```python
from build123d import *

# Parameters (mm, degrees)
SHAFT_PROFILE_6_R        = 3
SHAFT_6X95_DEPTH         = 47.5
HEAD_PROFILE_10_R        = 5
HEAD_10X5_DEPTH          = 5
HEAD_EDGE_FILLETS_R0_5_R = 0.5


with BuildPart() as part:
    # Shaft Profile Ø6 → Shaft Ø6x95 (new, symmetric)
    with BuildSketch(Plane.XY):
        Circle(SHAFT_PROFILE_6_R)
    extrude(amount=SHAFT_6X95_DEPTH, both=True)

    # Head Profile Ø10 → Head Ø10x5 (add)
    with BuildSketch(Plane.XY.offset(47.5)):
        Circle(HEAD_PROFILE_10_R)
    head_10x5 = extrude(amount=-HEAD_10X5_DEPTH)

    # Head Mirror: Head Ø10x5 across plane
    add(head_10x5.mirror(Plane.XY))

    # Head Edge Fillets R0.5
    head_edge_fillets_r0_5_edges = [part.edges().sort_by_distance(p)[0] for p in [
        (-3, 0, -42.5),
        (-5, 0, -47.5),
        (-3, 0, 42.5),
        (-5, 0, 47.5),
    ]]
    fillet(head_edge_fillets_r0_5_edges, radius=HEAD_EDGE_FILLETS_R0_5_R)


solid = part.part
```
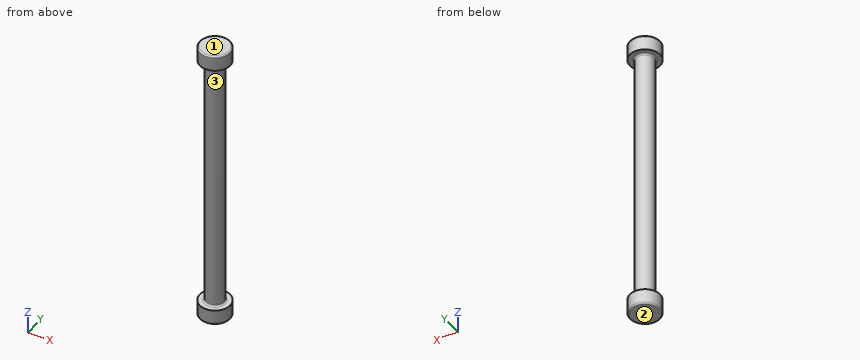
Here's how the part is built. I have some questions about the finished solid (model axes, mm). Face numbers are marked on the shaded views. Round coordinates to 2 decimals unless told otherwise and drop trailing zeros. Order: outer loops, then holes, each group sorted by start corner. A loop starts at its lowest first (then second) coordinate and runs counter-clockwise, first axis right, second up. Notation, with made-up numbers: M -21.5,4 L -15.5,4 A12 cw -15.5,12 Z; hole C 0.25,4.25 d7. An arc over 180 degrees is marked long. Answer as CSV lines item,"result".
Item 1: Imagine slicing it at C-C on z = -36. List the corners of the cut face in (x, y) for me.
From the geometry:
outline,"C 0,0 d6"
Item 2: We'd pull the mould along Z, two halves only. Please class the marked faces 1, 2 and 3: +Z half, -Z half, draft (parallel to the pull), parting line (faces both ways), or undercut.
From the geometry:
face 1,"+Z half"
face 2,"-Z half"
face 3,"undercut"
Item 3: Imagine slicing it at A-A on y = 0. List the corners of the cut face in (x, z) for me.
From the geometry:
outline,"M -5,-47 A0.5 ccw -4.5,-47.5 L 4.5,-47.5 A0.5 ccw 5,-47 L 5,-42.5 L 3.5,-42.5 A0.5 cw 3,-42 L 3,42 A0.5 cw 3.5,42.5 L 5,42.5 L 5,47 A0.5 ccw 4.5,47.5 L -4.5,47.5 A0.5 ccw -5,47 L -5,42.5 L -3.5,42.5 A0.5 cw -3,42 L -3,-42 A0.5 cw -3.5,-42.5 L -5,-42.5 Z"
Item 4: For pin 1 (4 mm diameter, centred on x = 1.5, z = -34.5, fed in from -Y); pin 2 (1.5 mm diameter, centred on x = 1, z = 18.5, fed in from +Y); pin 3 (1.5 mm diameter, centred on y = -1.5, z = 16, fed in from +X), each with a flat end and sliding along its axis, tell me the tip position at first contact or that it passes through.
From the geometry:
pin 1,"y = -3"
pin 2,"y = 2.99"
pin 3,"x = 2.9"
Item 5: Please list where these lines run through material, in increasing order: L1, parallel to Z at x = 3, y = -3.5; L2, parallel to Z at x = 3.25, y = 3.75; L3, parallel to Y at x = 0.25, z = -33.5. Write a range as [from, to].
From the geometry:
L1,"[-47.49, -42.5], [42.5, 47.49]"
L2,"[-47.19, -42.5], [42.5, 47.19]"
L3,"[-2.99, 2.99]"
